Print and shaded views of the part. All mm, measured from the part's lowest x, y and z. A direction names the side the tool comes from. Give positions to 0.01 mm unless a question says otherwise; leave off trailing zeros. Loops run counter-clockwise (first coordinate to the right, second up) from the corner with the lowest first, then second, coordinate; pieces in that order, holes last. Notation, with made-up numbers: M 22.5,-3.75 L 39.5,-3.75 A13 cw 39.5,14.25 Z; hole C -5,73.25 d11. An arc over 180 degrees is marked long. Put each result on its own line as item: value. Start each with the question number.
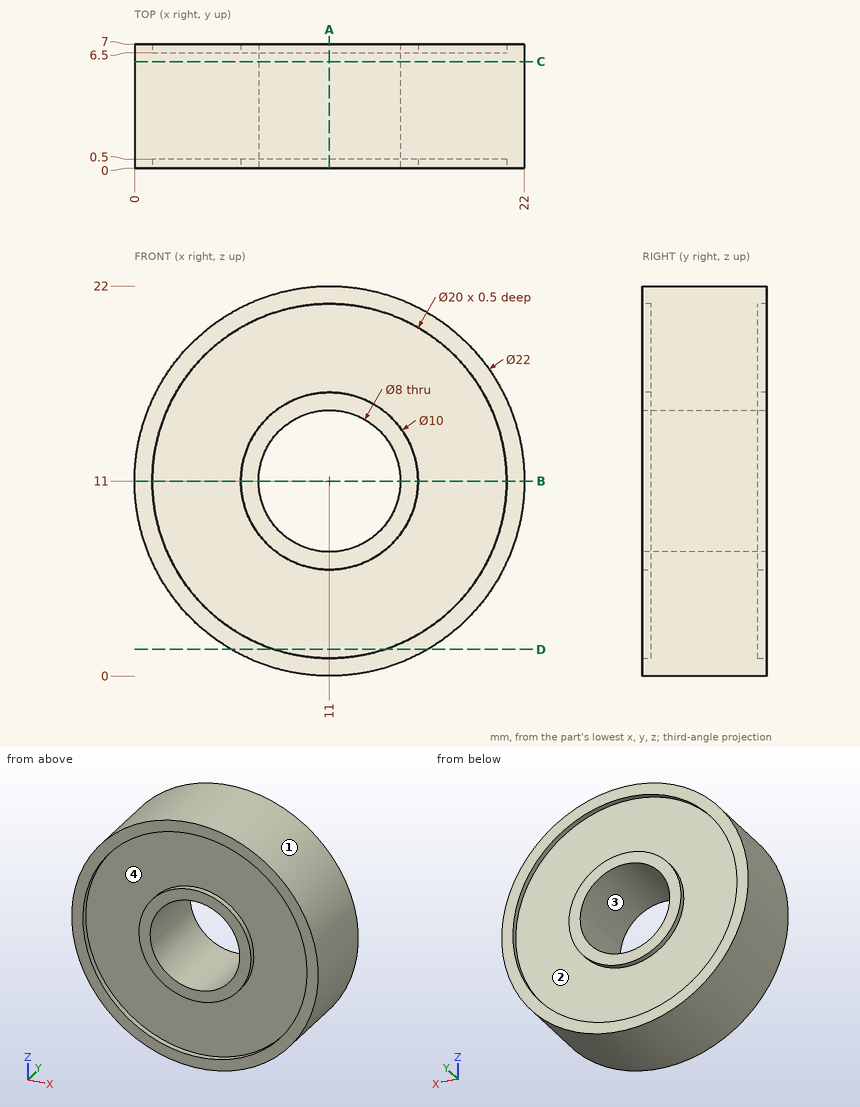
1) Wall check: L1, parallel to X at y = 0.35, z = 11; L2, parallel to X at y = 2.25, z = 11; L3, parallel to Y at x = 2.75, z = 16. Give the ranges that are in metal, low to high.
2) Mould opens along Z. For the marked faces 1 and 2 say: +Z half, -Z half, draft (parallel to the pull), parting line (faces both ways), or undercut.
3) Pin check, flat tips, straight feed: pin 1 Ø4 at (y, z) = (6, 2.5) entering from -X; pin 2 Ø1 at (x, y) = (16.5, 1.5) entering from -Z. Stop position of each tip, or through.
4) Band-saw the part on D-D on z = 1.5. Give the cut face in (x, y).
5) Band-saw the part on B-B on z = 11. Give the cut face in (x, y), then the cut area to 3 significant figures.
6) Which spindle directions (+Z, -Z, +X, -X, +Y, -Y) get a long thin tool onto all of the face, cutting with end or side? Do the marked faces 3 and 4. Say none if no direction does.
7) Band-saw the part on A-A on x = 11. Give the cut face in (y, z), then the cut area to 3 significant figures.
8) Band-saw the part on C-C on y = 6. Give the cut face in (x, z).
Evaluation:
1. L1: 0 to 1, 6 to 7, 15 to 16, 21 to 22
1. L2: 0 to 7, 15 to 22
1. L3: 0.5 to 6.5
2. face 1: parting line
2. face 2: undercut
3. pin 1: x = 2.13
3. pin 2: z = 1.2
4. outline: M 5.45,0 L 7.88,0 L 7.88,0.5 L 14.12,0.5 L 14.12,0 L 16.55,0 L 16.55,7 L 14.12,7 L 14.12,6.5 L 7.88,6.5 L 7.88,7 L 5.45,7 Z
5. outline: M 0,0 L 1,0 L 1,0.5 L 6,0.5 L 6,0 L 7,0 L 7,7 L 6,7 L 6,6.5 L 1,6.5 L 1,7 L 0,7 Z; M 15,0 L 16,0 L 16,0.5 L 21,0.5 L 21,0 L 22,0 L 22,7 L 21,7 L 21,6.5 L 16,6.5 L 16,7 L 15,7 Z
5. area: 88.0 mm2
6. face 3: +Y, -Y
6. face 4: -Y
7. outline: M 0,0 L 7,0 L 7,1 L 6.5,1 L 6.5,6 L 7,6 L 7,7 L 0,7 L 0,6 L 0.5,6 L 0.5,1 L 0,1 Z; M 0,15 L 7,15 L 7,16 L 6.5,16 L 6.5,21 L 7,21 L 7,22 L 0,22 L 0,21 L 0.5,21 L 0.5,16 L 0,16 Z
7. area: 88.0 mm2
8. outline: C 11,11 d22; hole C 11,11 d8
